Source: CAD feature listing. Evaluate the final solid. Frame: model axes, mm. A direction names the side the tool comes from. Coordinates: 2 decimals unless noted, no trailing zeros. Loops run counter-clockwise (first coordinate to the right, second up) from the corner with the lowest first, then second, coordinate; pieces in that order, holes last.
```python
from build123d import *

# Parameters (mm, degrees)
CUT_EXTRUDE1_DEPTH = 2
FILLET1_R          = 0.5
CHAMFER1_SIZE      = 0.1
CHAMFER1_SIZE2     = 0.567128182
CHAMFER2_SIZE      = 0.5


with BuildPart() as part:
    # Sketch1 → Revolve1 (revolve)
    with BuildSketch(Plane.XY, mode=Mode.PRIVATE) as revolve1_sk:
        Polygon((0, 0), (0, 3.5), (4, 3.5), (4, 2), (12, 2), (12, 0), align=None)
    revolve(revolve1_sk.sketch.rotate(Axis((-4.709244637, 0, 0), (1, 0, 0)), 90), axis=Axis((-4.709244637, 0, 0), (1, 0, 0)))

    # Sketch4 → Cut-Extrude1 (cut)
    with BuildSketch(Plane.ZY):
        Polygon((-1.732050808, 0), (-0.866025404, -1.5), (0.866025404, -1.5), (1.732050808, 0), (0.866025404, 1.5), (-0.866025404, 1.5), align=None)
    extrude(amount=-CUT_EXTRUDE1_DEPTH, mode=Mode.SUBTRACT)

    # Fillet1
    fillet1_edges = [part.edges().sort_by_distance(p)[0] for p in [
        (4, 0, -3.5),
        (0, 0, -3.5),
    ]]
    fillet(fillet1_edges, radius=FILLET1_R)

    # Chamfer1
    chamfer1_edges = [part.edges().sort_by_distance(p)[0] for p in [
        (0, 0.75, -1.299038106),
        (0, -0.75, -1.299038106),
        (0, -1.5, 0),
        (0, -0.75, 1.299038106),
        (0, 0.75, 1.299038106),
        (0, 1.5, 0),
    ]]
    chamfer1_side = [part.faces().sort_by_distance(p)[0] for p in [
        (0, 0, -2.915147186),
    ]]
    chamfer(chamfer1_edges, length=CHAMFER1_SIZE, length2=CHAMFER1_SIZE2, reference=chamfer1_side[0])

    # Chamfer2
    chamfer2_edges = [part.edges().sort_by_distance(p)[0] for p in [
        (12, 0, -2),
    ]]
    chamfer(chamfer2_edges, length=CHAMFER2_SIZE)


solid = part.part
```
Q1. Section query B-B on z = 0. Return the cut outline in (x, y).
Q2. Material intervals for line 1 along X through (y, z) = (-2, -2.25); line 2 along Y through (x, z) = (4.5, -1); line 3 along Y through (x, z) = (7.5, 0), sorted ascending.
Q3. Section query A-A on x = 1.25. Return the cut outline in (y, z), then the cut area to 3 significant figures.
Q4. Draft query along Y for faces 4 (the cylindrical face through (2.021, 3.105, 1.615)), 5 (the flat face through (4, 2, 1)), 6 (the flat face through (0.29, 0.76, 1.35)). Return one class per face: released by +Y, released by -Y, zero draft, split by the parting line, or undercut.
Q5. Reachability of faces 1 (the flat face through (2, 0, 0)), 2 (the flat face through (0, 1.3, -1.3)), 3 (the cylindrical face through (8, 2, 0)) from +Z, -Z, +X, -X, +Y, -Y: full face, straight path, thin tool, end or side. Return the list, or none.
Q6. First-contact query: pin 1 Ø1 at (x, z) = (8.5, 1) entering from +Y; pin 2 Ø3 at (x, y) = (4.5, -2) entering from -Z; pin 3 Ø0.9 at (y, z) = (0, 0) entering from -X; pin 4 Ø1.5 at (y, z) = (1, 0.5) entering from -X. Flat tips, straight axial feed; report the tip coordinate or a pass-through.
Resolved:
1. outline: (0, -3) arc R0.5 ccw to (0.5, -3.5) - (3.5, -3.5) arc R0.5 ccw to (4, -3) - (4, -2) - (11.5, -2) - (12, -1.5) - (12, 1.5) - (11.5, 2) - (4, 2) - (4, 3) arc R0.5 ccw to (3.5, 3.5) - (0.5, 3.5) arc R0.5 ccw to (0, 3) - (0, 1.6) - (0.57, 1.5) - (2, 1.5) - (2, -1.5) - (0.57, -1.5) - (0, -1.6) - close
2. line 1: x = 0 to 4
2. line 2: y = -1.73 to 1.73
2. line 3: y = -2 to 2
3. outline: circle Ø7 at (0, 0); hole (-1.5, -0.87) - (0, -1.73) - (1.5, -0.87) - (1.5, 0.87) - (0, 1.73) - (-1.5, 0.87) - close
3. area: 30.7 mm2
4. face 4: split by the parting line
4. face 5: zero draft
4. face 6: undercut
5. face 1: -X
5. face 2: +Z, -Z, -X, +Y, -Y
5. face 3: +X
6. pin 1: stops at y = 1.94
6. pin 2: stops at z = -3.4
6. pin 3: stops at x = 2
6. pin 4: stops at x = 0
